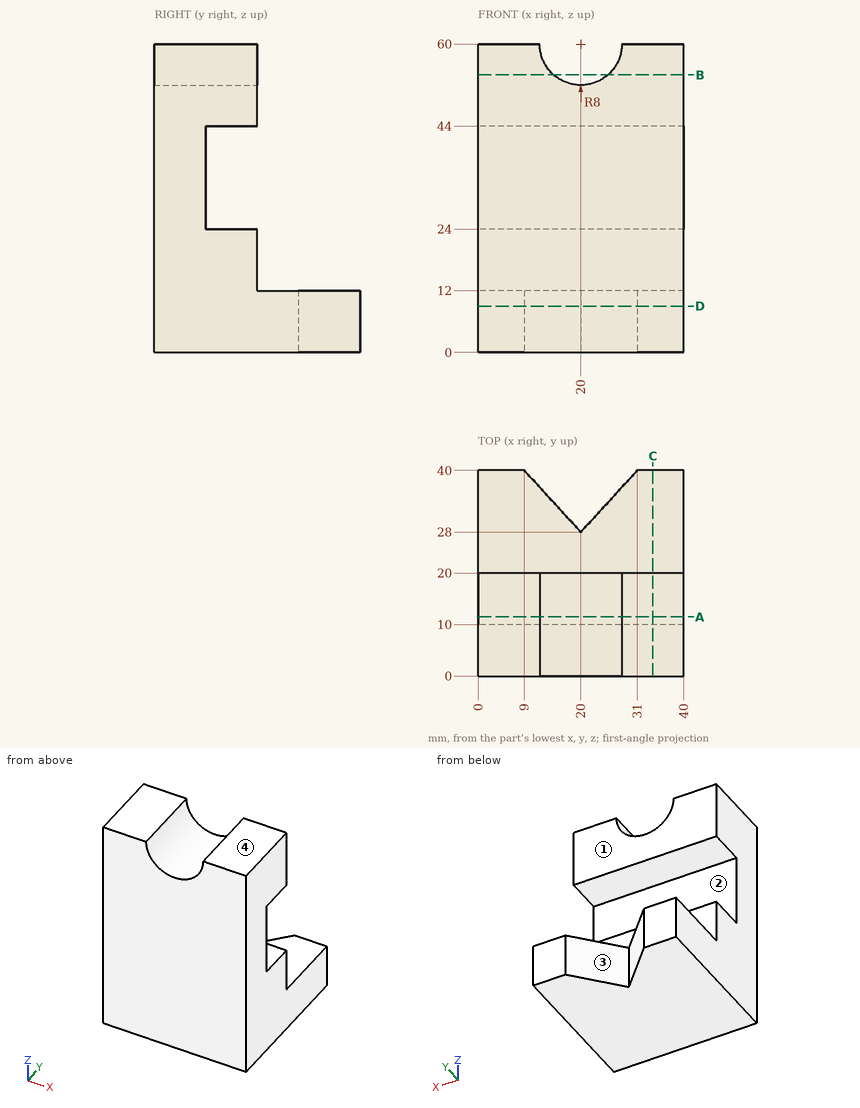
Geometry check sheet. Reference: drawing and pictorial views, mm from the part's lowest x, y, z. A direction names the side the tool comes from. Round coordinates to 2 decimals unless told otherwise and drop trailing zeros. Order: outer loops, then holes, each group sorted by start corner. A loop starts at its lowest first (then second) coordinate and runs counter-clockwise, first axis right, second up. Notation, with made-up numbers: M 13.5,-34.75 L 20.5,-34.75 A19 cw 20.5,-8.75 Z; hole C 30,-25.75 d8. An arc over 180 degrees is marked long. Answer in a Markdown table with one row per item.
(1) Go/stop test with flat-tipped pins: P1, Ø3, axis at x = 21, y = 13, coming from the -Z side; P2, Ø13, axis at x = 17.5, z = 51.5, coming from the +Y side; P3, Ø5, axis at x = 21, y = 8.5, coming from the +Z side; P4, Ø5, axis at x = 16.5, y = 22, coming from the +Z side (3 decimals). Record where each tip stops, or that it passes through.
Responses:
| item | result |
|---|---|
| P1 | stops at z = 0 |
| P2 | stops at y = 20 |
| P3 | stops at z = 52.81 |
| P4 | stops at z = 53.755 |
(2) Tool access check on the marked faces 1, 2, 3 and 4. Record the directions out of +Z, -Z, +X, -X, +Y, -Y that give a thin tool (end or side, any length) a straight path to the whole face; none if there is none.
Responses:
| item | result |
|---|---|
| face 1 | +Z, +X, -X, +Y |
| face 2 | +X, -X, +Y |
| face 3 | +Z, -Z, +Y |
| face 4 | +Z, +X, -X, +Y, -Y |
(3) Scan lines: probe 1 along Z at (x, y) = (36.5, 13.5); probe 2 along Z at (x, y) = (37, 31); probe 3 along Y at (x, z) = (21, 27). Record each from-to range of solid material in increasing order. Write a range as from..to.
Responses:
| item | result |
|---|---|
| probe 1 | z = 0..24, 44..60 |
| probe 2 | z = 0..12 |
| probe 3 | y = 0..10 |
(4) Sectioned sample at A-A, the plane y = 11.5. Record the cut outline in (x, z), and give its area (3 significant figures).
Responses:
| item | result |
|---|---|
| outline | M 0,0 L 40,0 L 40,24 L 0,24 Z; M 0,44 L 40,44 L 40,60 L 28,60 A8 cw 12,60 L 0,60 Z |
| area | 1,500 mm² |
(5) Sectioned sample at D-D, the plane z = 9. Record the cut outline in (x, y).
Responses:
| item | result |
|---|---|
| outline | M 0,0 L 40,0 L 40,40 L 31,40 L 20,28 L 9,40 L 0,40 Z |
(6) Sectioned sample at C-C, the plane x = 34. Record the cut outline in (y, z).
Responses:
| item | result |
|---|---|
| outline | M 0,0 L 40,0 L 40,12 L 20,12 L 20,24 L 10,24 L 10,44 L 20,44 L 20,60 L 0,60 Z |
(7) Sectioned sample at B-B, the plane z = 54. Record the cut outline in (x, y).
Responses:
| item | result |
|---|---|
| outline | M 0,0 L 14.71,0 L 14.71,20 L 0,20 Z; M 25.29,0 L 40,0 L 40,20 L 25.29,20 Z |
